from build123d import *

# Parameters (mm, degrees)
CUT_EXTRUDE1_REACH = 42.893
SKETCH2_W          = 1
SKETCH2_H          = 9.301452206
SKETCH2_H_2        = 8.508093048
CHAMFER2_SIZE      = 0.3


with BuildPart() as part:
    # Sketch1 → Revolve1 (revolve)
    with BuildSketch(Plane.XY, mode=Mode.PRIVATE) as revolve1_sk:
        Polygon((0, 0), (40.5, 0), (40.5, 1.9), (34.5, 1.9), (34.5, 2), (23, 2), (23, 3), (10, 3), (10, 4), (0, 4), align=None)
    revolve(revolve1_sk.sketch.rotate(Axis((0, 0, 0), (1, 0, 0)), 90), axis=Axis((0, 0, 0), (1, 0, 0)))

    # Sketch2 → Cut-Extrude1 (cut, up to next)
    with BuildSketch(Plane.ZY, mode=Mode.PRIVATE) as cut_extrude1_sk1:
        with Locations((-3.5, 0)):
            Rectangle(SKETCH2_W, SKETCH2_H)
    cut_extrude1_tool1 = extrude(cut_extrude1_sk1.sketch, amount=-CUT_EXTRUDE1_REACH, mode=Mode.PRIVATE) & part.part
    # Sketch2 → Cut-Extrude1 (cut, up to next)
    with BuildSketch(Plane.ZY, mode=Mode.PRIVATE) as cut_extrude1_sk2:
        with Locations((3.5, 0)):
            Rectangle(SKETCH2_W, SKETCH2_H_2)
    cut_extrude1_tool2 = extrude(cut_extrude1_sk2.sketch, amount=-CUT_EXTRUDE1_REACH, mode=Mode.PRIVATE) & part.part
    add(cut_extrude1_tool1.solids().sort_by_distance((0, 0, -3.5))[0], mode=Mode.SUBTRACT)
    add(cut_extrude1_tool2.solids().sort_by_distance((0, 0, 3.5))[0], mode=Mode.SUBTRACT)

    # Chamfer2
    chamfer2_edges = [part.edges().sort_by_distance(p)[0] for p in [
        (23, 0, -3),
        (0, 4, 0),
        (0, -4, 0),
        (0, 0, -3),
        (0, 0, 3),
        (40.5, 0, -1.9),
    ]]
    chamfer(chamfer2_edges, length=CHAMFER2_SIZE)


solid = part.part
Model file for the job. Use its own axes, mm. A direction names the side the tool comes from. Give positions to 0.01 mm unless a question says otherwise; leave off trailing zeros. Loops run counter-clockwise (first coordinate to the right, second up) from the corner with the lowest first, then second, coordinate; pieces in that order, holes last.
Item 1: Slice it at C-C (x = 24). Write the cut outline in (y, z), plus the area to 3 significant figures.
Check values:
outline: circle Ø4 at (0, 0)
area: 12.6 mm2
Item 2: Drop flat-ended pins along their axis: P1, Ø1, axis at x = 22.5, z = 1, coming from the -Y side; P2, Ø1.2, axis at y = -2.5, z = -1, coming from the +X side; P3, Ø1.2, axis at y = 2.5, z = -0.5, coming from the +X side. Give the stop position or say it passes through.
Check values:
P1: stops at y = -2.96
P2: stops at x = 23
P3: stops at x = 34.5
Item 3: Slice it at A-A (z = 0). Write the cut outline in (x, y).
Check values:
outline: (0, -3.7) - (0.3, -4) - (10, -4) - (10, -3) - (22.7, -3) - (23, -2.7) - (23, -2) - (34.5, -2) - (34.5, -1.9) - (40.2, -1.9) - (40.5, -1.6) - (40.5, 1.6) - (40.2, 1.9) - (34.5, 1.9) - (34.5, 2) - (23, 2) - (23, 2.7) - (22.7, 3) - (10, 3) - (10, 4) - (0.3, 4) - (0, 3.7) - close
Item 4: Slice it at B-B (x = 4). Write the cut outline in (y, z), plus the area to 3 significant figures.
Check values:
outline: (-2.65, -3) - (2.65, -3) arc R4 ccw to (2.65, 3) - (-2.65, 3) arc R4 ccw to start
area: 43.0 mm2
Item 5: Drill centre lines: line 1 along X through (y, z) = (1.5, 1.75); line 2 along X through (y, z) = (-3.5, -1); line 3 along Y through (x, z) = (6, -1.75). Where is each one in solid material? Low to high.
Check values:
line 1: x = 0 to 23
line 2: x = 0 to 10
line 3: y = -3.6 to 3.6
Item 6: Which spindle directions (+Z, -Z, +X, -X, +Y, -Y) get a long thin tool onto all of the face, cutting with end or side? Do faces 1 (the face through (29, 2, 0)), 2 (the face through (10, -3.2, -0.2)), 3 (the face through (10, 3.2, -0.2)). Say none if no direction does.
Check values:
face 1: +X
face 2: +X, -Y
face 3: +X, +Y
